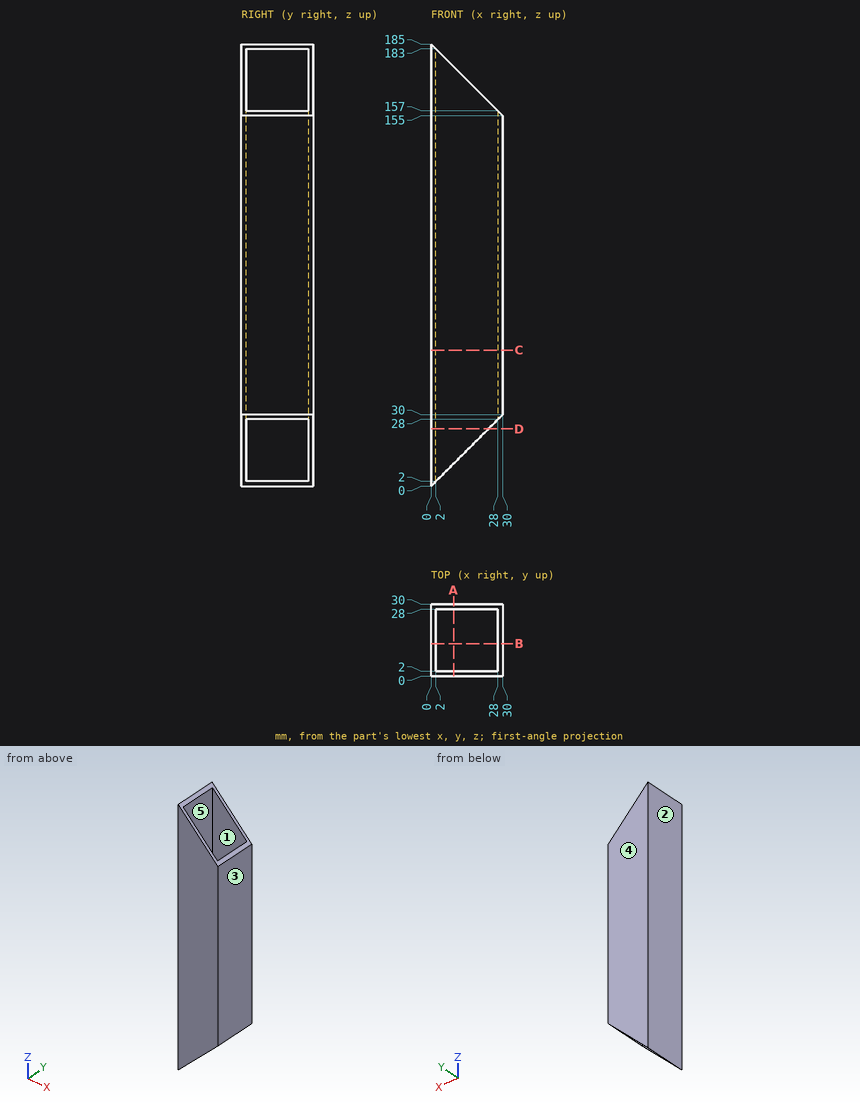
Verification items for this drawing (mm, ordinates from the low corner). A direction names the side the tool comes from. Coordinates: 2 decimals unless noted, no trailing zeros. Order: outer loops, then holes, each group sorted by start corner. A loop starts at its lowest first (then second) coordinate and runs counter-clockwise, first axis right, second up. Notation, with made-up numbers: M 83.5,-39 L 124.5,-39 A17 cw 124.5,-22 Z; hole C 5.5,-25 d7. An arc over 180 degrees is marked long. Write each question's results on one line, items separated by ' | '.
1) Access from +Z, -Z, +X, -X, +Y, -Y to the whole of each face (thin tool, end or side, straight path). Record for the marked faces 1 and 2.
Solved:
face 1: +Z, -Z | face 2: +Z, -Z, -X, +Y, -Y
2) Scan lines: line 1 along Y through (x, z) = (3, 89); line 2 along X through (y, z) = (11, 8). Record each from-to range of solid material in increasing order. Write a range as [from, to].
Solved:
line 1: y = [0, 2], [28, 30] | line 2: x = [0, 2]
3) Section check D-D on z = 24. Record the cut outline in (x, y), plus the area to 3 significant figures.
Solved:
outline: M 0,0 L 24,0 L 24,2 L 2,2 L 2,28 L 24,28 L 24,30 L 0,30 Z | area: 148 mm²
4) Section check C-C on z = 57. Record the cut outline in (x, y).
Solved:
outline: M 0,0 L 30,0 L 30,30 L 0,30 Z; hole M 2,2 L 28,2 L 28,28 L 2,28 Z
5) Section check A-A on x = 9.5. Record the cut outline in (y, z).
Solved:
outline: M 0,9.5 L 2,9.5 L 2,175.5 L 0,175.5 Z; M 28,9.5 L 30,9.5 L 30,175.5 L 28,175.5 Z
6) Gauge pin test, flat ends, axial feed: pin 1 Ø4 at (x, y) = (10, 26.5) entering from -Z; pin 2 Ø8 at (y, z) = (12, 23) entering from +X; pin 3 Ø12 at (x, y) = (17.5, 3) entering from -Z; pin 4 Ø1 at (x, y) = (9, 26.5) entering from -Z. Record the tip position at first contact, or that the pin passes through.
Solved:
pin 1: stops at z = 8.68 | pin 2: stops at x = 2 | pin 3: stops at z = 11.58 | pin 4: passes through
7) Section check B-B on y = 13.5. Record the cut outline in (x, z).
Solved:
outline: M 0,0 L 2,2 L 2,183 L 0,185 Z; M 28,28 L 30,30 L 30,155 L 28,157 Z
8) Release check for a two-part mould opening along Y. For the marked faces 3, 4 and 5 record: pulls with the +Y half, pulls with the -Y half, needs draft (parallel to the pull), parting line crosses it, or undercut.
Solved:
face 3: needs draft | face 4: pulls with the +Y half | face 5: undercut
